Verification items for the finished model (mm, model axes). A direction names the side the tool comes from. Round coordinates to 2 decimals unless told otherwise and drop trailing zeros. Write each loop counter-clockwise with the first axis right and the second up, starting at its lowest first coordinate (ties: lowest second). Pieces come first, ordered by that corner, then holes.
from build123d import *

# Parameters (mm, degrees)
SKETCH1_R           = 11
BOSS_EXTRUDE1_DEPTH = 10.5
SKETCH2_OUTSIDE_W   = 30.568
SKETCH2_OUTSIDE_H   = 30.568
SKETCH2_OUTSIDE_R   = 5
CUT_EXTRUDE1_DEPTH  = 2.4
SKETCH3_R           = 4
CUT_EXTRUDE2_DEPTH  = 4.15
SKETCH4_R           = 8.75
CUT_EXTRUDE3_DEPTH  = 3
CHAMFER1_SIZE       = 0.2


with BuildPart() as part:
    # Sketch1 → Boss-Extrude1 (new body)
    with BuildSketch(Plane.XY):
        with Locations(Location((0, 0, 0), (0, 0, 180))):
            Circle(SKETCH1_R)
    extrude(amount=BOSS_EXTRUDE1_DEPTH)

    # Sketch2 outside → Cut-Extrude1 (cut)
    with BuildSketch(Plane.XY.offset(10.5)):
        Rectangle(SKETCH2_OUTSIDE_W, SKETCH2_OUTSIDE_H)
        Circle(SKETCH2_OUTSIDE_R, mode=Mode.SUBTRACT)
    extrude(amount=-CUT_EXTRUDE1_DEPTH, mode=Mode.SUBTRACT)

    # Sketch3 → Cut-Extrude2 (cut)
    with BuildSketch(Plane.XY.offset(10.5)):
        Circle(SKETCH3_R)
    extrude(amount=-CUT_EXTRUDE2_DEPTH, mode=Mode.SUBTRACT)

    # Sketch4 → Cut-Extrude3 (cut)
    with BuildSketch(Plane(origin=(0, 0, 0), x_dir=(-1, 0, 0), z_dir=(0, 0, -1))):
        Circle(SKETCH4_R)
    extrude(amount=-CUT_EXTRUDE3_DEPTH, mode=Mode.SUBTRACT)

    # Chamfer1
    chamfer1_edges = [part.edges().sort_by_distance(p)[0] for p in [
        (8.75, 0, 0),
    ]]
    chamfer(chamfer1_edges, length=CHAMFER1_SIZE)


solid = part.part
Q1. Sectioned sample at D-D (y = -9.5). Enter the section's corners in (x, z).
Recorded:
outline: (-5.55, 0) - (5.55, 0) - (5.55, 8.1) - (-5.55, 8.1) - close
Q2. Tool access check on faces 1 (the cylindrical face through (2.38, 10.74, 3.99)), 2 (the flat face through (0, 0, 3)). Record the directions out of +Z, -Z, +X, -X, +Y, -Y that give a thin tool (end or side, any length) a straight path to the whole face; none if there is none.
Recorded:
face 1: +Z, -Z
face 2: -Z
Q3. Sectioned sample at B-B (z = 2.25). Enter the section's corners in (x, y), plus the area to 3 significant figures.
Recorded:
outline: circle Ø22 at (0, 0); hole circle Ø17.5 at (0, 0)
area: 140 mm2
Q4. Material ranges on line 1 along Y through (x, z) = (0, 1.75); line 2 along Z through (x, y) = (6.25, -4.75); line 3 along Z through (x, y) = (-3.75, -9.5), recorded low to high.
Recorded:
line 1: y = -11 to -8.75, 8.75 to 11
line 2: z = 3 to 8.1
line 3: z = 0 to 8.1
Q5. Sectioned sample at C-C (z = 5). Enter the section's corners in (x, y), plus the area to 3 significant figures.
Recorded:
outline: circle Ø22 at (0, 0)
area: 380 mm2
Q6. Sectioned sample at A-A (x = 0). Enter the section's corners in (y, z).
Recorded:
outline: (-11, 0) - (-8.95, 0) - (-8.75, 0.2) - (-8.75, 3) - (8.75, 3) - (8.75, 0.2) - (8.95, 0) - (11, 0) - (11, 8.1) - (5, 8.1) - (5, 10.5) - (4, 10.5) - (4, 6.35) - (-4, 6.35) - (-4, 10.5) - (-5, 10.5) - (-5, 8.1) - (-11, 8.1) - close
Q7. Release check for a two-part mould opening along Y. For faces 3 (the cylindrical face through (-0.867, -3.905, 8.454)), 4 (the flat face through (0, 0, 6.35)), 5 (the cylindrical face through (-1.08, -4.88, 9.32)), 6 (the flat face through (2, -5, 8.1)) record: released by +Y, released by -Y, zero draft, split by the parting line, or undercut.
Recorded:
face 3: undercut
face 4: undercut
face 5: split by the parting line
face 6: zero draft
Q8. Depth check by flat-ended pin: P1, Ø5, axis at x = 3, y = 3, coming from the -Z side; P2, Ø1.5, axis at y = 1, z = 5, coming from the -X side; P3, Ø1.5, axis at x = -5, z = 3.5, coming from the -Y side. Enter the tip coordinate at first touch or a pass-through.
Recorded:
P1: stops at z = 3
P2: stops at x = -11
P3: stops at y = -10.15
